from build123d import *

# Parameters (mm, degrees)
EXTRUDE1_DEPTH      = 9
EXTRUDE1_DEPTH_BACK = 9


with BuildPart() as part:
    # Sketch1 → Extrude1 (new, two sides: drawn at the far end of the back side and taken through both)
    with BuildSketch(Plane(origin=(0, 0, 0), x_dir=(0, 0, -1), z_dir=(1, 0, 0)).offset(-EXTRUDE1_DEPTH_BACK)):
        Polygon((0, -31.754264805), (27.5, -15.877132403), (27.5, 15.877132403), (0, 31.754264805), (-27.5, 15.877132403), (-27.5, -15.877132403), align=None)
    extrude(amount=EXTRUDE1_DEPTH + EXTRUDE1_DEPTH_BACK)

    # Sketch4 → M36x2.0 Tapped Hole1 (revolve, cut)
    with BuildSketch(Plane(origin=(-9, 0, 0), x_dir=(0, 0, 1), z_dir=(0, 1, 0))):
        Polygon((0, 0), (0, 88.214630523), (17, 78), (17, 72), (18, 72), (18, 0), align=None)
    revolve(axis=Axis((-15.35, 0, 0), (1, 0, 0)), mode=Mode.SUBTRACT)

    # Sketch2 → Cut-Revolve1 (revolve, cut)
    with BuildSketch(Plane.XY, mode=Mode.PRIVATE) as cut_revolve1_sk:
        Polygon((9, 31.754264805), (6.113248654, 31.754264805), (9, 26.754264805), align=None)
    cut_revolve1 = revolve(cut_revolve1_sk.sketch.rotate(Axis((-9, 0, 0), (-1, 0, 0)), 240.000000138), axis=Axis((-9, 0, 0), (-1, 0, 0)), mode=Mode.SUBTRACT)

    # Mirror1: Cut-Revolve1 across plane
    add(cut_revolve1.mirror(Plane(origin=(0, 0, 0), x_dir=(0, 0, 1), z_dir=(1, 0, 0))), mode=Mode.SUBTRACT)


solid = part.part
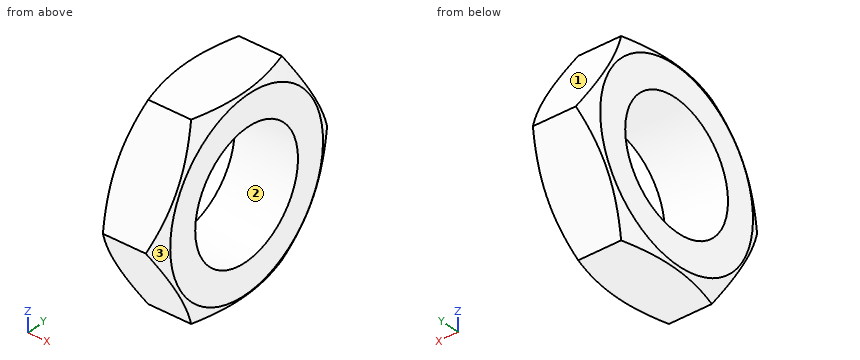
The listing builds one solid part. Answer for the finished solid, in the listing's coordinates (mm). Face numbers are marked on the shaded views. Give positions to 0.01 mm unless a question says otherwise; leave off trailing zeros. Order: outer loops, then holes, each group sorted by start corner. A loop starts at its lowest first (then second) coordinate and runs counter-clockwise, first axis right, second up. Notation, with made-up numbers: (59.25, 69.25) - (84.25, 69.25) arc R23 ccw to (84.25, 90.25) - close; hole circle Ø6 at (56, 88.25). An arc over 180 degrees is marked (long way). Answer as CSV lines item,"result".
Q1. A cutting plane is placed at A-A, the plane x = 3.25. Determine the outline of the cut face in (y, z), and give its area (3 significant figures).
Answer key:
outline,"(-31.75, 0) - (-15.88, -27.5) - (15.88, -27.5) - (31.75, 0) - (15.88, 27.5) - (-15.88, 27.5) - close; hole circle Ø36 at (0, 0)"
area,"1,600 mm^2"
Q2. A cutting plane is placed at B-B, the plane y = 0. Determine the outline of the cut face in (x, z).
Answer key:
outline,"(-9, -26.75) - (-8.57, -27.5) - (8.57, -27.5) - (9, -26.75) - (9, -18) - (-9, -18) - close; (-9, 18) - (9, 18) - (9, 26.75) - (8.57, 27.5) - (-8.57, 27.5) - (-9, 26.75) - close"
Q3. Determine the mould class of the marked faces 1, 2 and 3 for opening direction Y: pulls with the +Y half, pulls with the -Y half, needs draft (parallel to the pull), parting line crosses it, or undercut.
Answer key:
face 1,"pulls with the +Y half"
face 2,"undercut"
face 3,"parting line crosses it"
Q4. A cutting plane is placed at C-C, the plane x = 7. Determine the outline of the cut face in (y, z), and give its area (3 significant figures).
Answer key:
outline,"(-30.08, -2.9) - (-17.55, -24.6) arc R30.22 ccw to (-12.53, -27.5) - (12.53, -27.5) arc R30.22 ccw to (17.55, -24.6) - (30.08, -2.9) arc R30.22 ccw to (30.08, 2.9) - (17.55, 24.6) arc R30.22 ccw to (12.53, 27.5) - (-12.53, 27.5) arc R30.22 ccw to (-17.55, 24.6) - (-30.08, 2.9) arc R30.22 ccw to start; hole circle Ø36 at (0, 0)"
area,"1,580 mm^2"
Q5. Each of these flat-tipped pins is pushed along its axis until it touches: pin 1 Ø3 at (x, z) = (-3.5, -16) entering from -Y; pin 2 Ø2 at (x, z) = (0.5, -8.5) entering from -Y; pin 3 Ø10 at (x, z) = (5.5, -18.5) entering from +Y; pin 4 Ø3 at (y, z) = (24.5, 17) entering from -X. Where does it stop, or does it pass through?
Answer key:
pin 1,"stops at y = -23.38"
pin 2,"stops at y = -27.42"
pin 3,"stops at y = 23.96"
pin 4,"passes through"
Q6. Straight lines are drawn through the part: L1, parallel to Z at x = 1.5, y = 0; L2, parallel to Y at x = 8.25, z = 0; L3, parallel to Y at x = 4, z = -8. For each, find the intervals that lie inside material, in ascending order.
Answer key:
L1,"z = -27.5 to -18, 18 to 27.5"
L2,"y = -28.05 to -18, 18 to 28.05"
L3,"y = -27.14 to -16.12, 16.12 to 27.14"
